Geometry: final body of the model. Coordinates: model frame, mm. A direction names the side the tool comes from. Coordinates: 2 decimals unless noted, no trailing zeros. Loops run counter-clockwise (first coordinate to the right, second up) from the corner with the lowest first, then second, coordinate; pieces in that order, holes last. Notation, with made-up numbers: (-26.75, 59.5) -> (20.25, 59.5) arc R14 cw to (20.25, 71.5) -> close; hole circle Ø6 at (-11.5, -6.75). An arc over 180 degrees is marked (long way). One line per item, written item: value. Start each with the question number.
Item 1: Section query B-B on z = 9.5. Return loops of the section in (x, y), then the cut area to 3 significant figures.
Item 2: Set-up query: faces 1 (the flat face through (-5, 0, -5)), 2 (the flat face through (-15.9, -25.4, 20.3)). Return all of +Z, -Z, +X, -X, +Y, -Y with unobstructed straight access to the full face (end or side cutting, diameter ignored); none if empty.
Item 3: Section query A-A on y = 3.5. Return loops of the section in (x, z), then the cut area to 3 significant figures.
Item 4: Section query C-C on x = -37.5. Return loops of the section in (y, z), then the cut area to 3 significant figures.
Item 5: Contact query for flat-ended pins moving along their axis: pin 1 Ø5 at (y, z) = (4, 8.5) entering from -X; pin 2 Ø8 at (x, y) = (-7.5, 8) entering from -Z. Output: stop coordinate, or through.
Item 6: Ray query, probe 1 along Z at (x, y) = (-31.5, -13); probe 2 along X at (y, z) = (3.5, 5); probe 3 along X at (y, z) = (2.5, 21). Return the intervals inside material, ascending. Write a range as from..to.
from build123d import *

# Parameters (mm, degrees)
EXTRUDE1_DEPTH = 25.4
FILLET1_R      = 5.5
FILLET2_R      = 1.67


with BuildPart() as part:
    # Sketch1 → Extrude1 (new, symmetric)
    with BuildSketch(Plane(origin=(0, 0, 0), x_dir=(1, 0, 0), z_dir=(0, 1, 0))):
        Polygon((0, -25), (0, 25), (-5, 25), (-5, -20), (-50, -20), (-50, -25), align=None)
    extrude(amount=EXTRUDE1_DEPTH, both=True)

    # Fillet1
    fillet1_edges = [part.edges().sort_by_distance(p)[0] for p in [
        (-5, 0, 20),
    ]]
    fillet(fillet1_edges, radius=FILLET1_R)

    # Fillet2
    fillet2_edges = [part.edges().sort_by_distance(p)[0] for p in [
        (-50, 0, 20),
        (-5, 0, -25),
    ]]
    fillet(fillet2_edges, radius=FILLET2_R)


solid = part.part
Reply:
1. outline: (-5, -25.4) -> (0, -25.4) -> (0, 25.4) -> (-5, 25.4) -> close
1. area: 254 mm²
2. face 1: -Z, -X, +Y, -Y
2. face 2: +Z, -Z, +X, -X, -Y
3. outline: (-50, 21.67) arc R1.67 ccw to (-48.33, 20) -> (-10.5, 20) arc R5.5 cw to (-5, 14.5) -> (-5, -23.33) arc R1.67 ccw to (-3.33, -25) -> (0, -25) -> (0, 25) -> (-50, 25) -> close
3. area: 480 mm²
4. outline: (-25.4, 20) -> (25.4, 20) -> (25.4, 25) -> (-25.4, 25) -> close
4. area: 254 mm²
5. pin 1: stops at x = -5
5. pin 2: stops at z = -24.99
6. probe 1: z = 20..25
6. probe 2: x = -5..0
6. probe 3: x = -49.86..0
